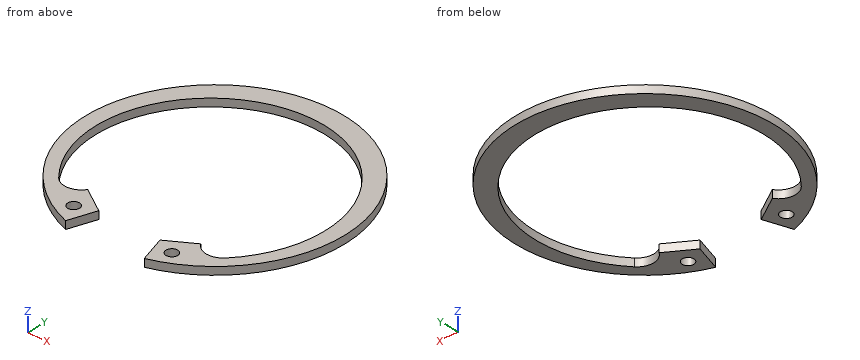
from build123d import *

# Parameters (mm, degrees)
BASE_EXTRUDE_DEPTH      = 1
BASE_EXTRUDE_DEPTH_BACK = 1
SKETCH1_R               = 1.5


with BuildPart() as part:
    # Sketch1 → Base-Extrude (new, two sides: drawn at the far end of the back side and taken through both)
    with BuildSketch(Plane.XY.offset(-BASE_EXTRUDE_DEPTH_BACK)):
        with BuildLine():
            Line((-14.724384167, -20.222967583), (-7.957187605, -24.489705295))
            Line((-7.957187605, -24.489705295), (-10.228462514, -31.479970689))
            ThreePointArc((-10.228462514, -31.479970689), (0, 33.1), (10.228462514, -31.479970689))
            Line((10.228462514, -31.479970689), (7.957187605, -24.489705295))
            Line((7.957187605, -24.489705295), (14.724384167, -20.222967583))
            ThreePointArc((14.724384167, -20.222967583), (18.073876023, -22.260468599), (21.719080421, -20.817211524))
            ThreePointArc((21.719080421, -20.817211524), (0, 27.9), (-21.719080421, -20.817211524))
            ThreePointArc((-21.719080421, -20.817211524), (-18.073876023, -22.260468599), (-14.724384167, -20.222967583))
        make_face()
        with Locations((-12.773653929, -26.368992497)):
            Circle(SKETCH1_R, mode=Mode.SUBTRACT)
        with Locations(Location((12.773653929, -26.368992497, 0), (0, 0, 180))):
            Circle(SKETCH1_R, mode=Mode.SUBTRACT)
    extrude(amount=BASE_EXTRUDE_DEPTH + BASE_EXTRUDE_DEPTH_BACK)


solid = part.part
Build history of the part. All positions in model axes, mm. Give positions to 0.01 mm unless a question says otherwise; leave off trailing zeros. Loops run counter-clockwise (first coordinate to the right, second up) from the corner with the lowest first, then second, coordinate; pieces in that order, holes last. Notation, with made-up numbers: (-4, -5) -> (54, -5) arc R25 ccw to (54, 15) -> close; hole circle Ø1 at (62.25, 42). An arc over 180 degrees is marked (long way). Answer in a Markdown table with one row per item.
Item 1: Slice it at C-C on z = 0.2. Write the cut outline in (x, y), plus the area to 3 significant figures.
Findings below:
| item | result |
|---|---|
| outline | (-21.72, -20.82) arc R29.2 cw (long way) to (21.72, -20.82) arc R4.4 cw to (14.72, -20.22) -> (7.96, -24.49) -> (10.23, -31.48) arc R33.1 ccw (long way) to (-10.23, -31.48) -> (-7.96, -24.49) -> (-14.72, -20.22) arc R4.4 cw to start; hole circle Ø3 at (-12.77, -26.37); hole circle Ø3 at (12.77, -26.37) |
| area | 799 mm² |
Item 2: Slice it at B-B on x = -23. Write the cut outline in (y, z), plus the area to 3 significant figures.
Findings below:
| item | result |
|---|---|
| outline | (-23.8, -1) -> (-19.29, -1) -> (-19.29, 1) -> (-23.8, 1) -> close; (16.69, -1) -> (23.8, -1) -> (23.8, 1) -> (16.69, 1) -> close |
| area | 23.3 mm² |
Item 3: Flat gauge pins, fed straight in: P1, Ø4, axis at x = -12.77, y = -26.37, coming from the +Z side; P2, Ø1, axis at y = -19.5, z = 0, coming from the +X side; P3, Ø1, axis at y = -22, z = 0.5, coming from the -X side. Where does each tip first touch, or does it go through?
Findings below:
| item | result |
|---|---|
| P1 | stops at z = 1 |
| P2 | stops at x = 27.1 |
| P3 | stops at x = -25.17 |
Item 4: Probe line 1 along X through (y, z) = (-26.5, 0.05); line 2 along Y through (x, z) = (11.5, -0.15); line 3 along Y through (x, z) = (-17, 0). List the from-to ranges inside material, lowest first. Write a range as [from, to].
Findings below:
| item | result |
|---|---|
| line 1 | x = [-19.83, -14.27], [-11.28, -8.61], [8.61, 11.28], [14.27, 19.83] |
| line 2 | y = [-31.04, -27.16], [-25.58, -22.26], [25.54, 31.04] |
| line 3 | y = [-28.4, -22.03], [22.44, 28.4] |
Item 5: Slice it at A-A on y = -1.3. Write the cut outline in (x, z).
Findings below:
| item | result |
|---|---|
| outline | (-33.07, -1) -> (-29.2, -1) -> (-29.2, 1) -> (-33.07, 1) -> close; (29.2, -1) -> (33.07, -1) -> (33.07, 1) -> (29.2, 1) -> close |
Item 6: Slice it at D-D on x = 0. Write the cut outline in (y, z).
Findings below:
| item | result |
|---|---|
| outline | (27.9, -1) -> (33.1, -1) -> (33.1, 1) -> (27.9, 1) -> close |
